Input: part model. Units: mm. Frame: model coordinates. A direction names the side the tool comes from. Coordinates: 2 decimals unless noted, no trailing zeros. Order: outer loops, then holes, each group sorted by start corner. A loop starts at its lowest first (then second) coordinate and runs counter-clockwise, first axis right, second up. Notation, with made-up numbers: (80.25, 5) -> (97.25, 5) arc R22 ccw to (97.25, 16) -> close; hole circle Ø2 at (78.25, 62.25). An arc over 180 degrees is marked (long way). Answer as CSV lines item,"result".
from build123d import *

# Parameters (mm, degrees)
SKETCH_1_R              = 19.5
EXTRUDE_1_DEPTH         = 25
CUT_EXTRUDE_1_DEPTH     = 5.95
SKETCH_3_R              = 20
EXTRUDE_2_DEPTH         = 21
SKETCH_4_R              = 23
EXTRUDE_3_DEPTH         = 150
CUT_EXTRUDE_START       = -30
CUT_EXTRUDE_2_DEPTH     = 30
HOLE_WIZARD_M10_1_D     = 8.5
HOLE_WIZARD_M10_1_DEPTH = 20
HOLE_WIZARD_M10_1_TIP   = 2.553657631


with BuildPart() as part:
    # 草图1 → 凸台-拉伸1 (new body)
    with BuildSketch(Plane(origin=(0, 0, 0), x_dir=(0, 0, -1), z_dir=(1, 0, 0))):
        Circle(SKETCH_1_R)
    extrude(amount=EXTRUDE_1_DEPTH)

    # 草图2 → 切除-拉伸1 (cut)
    with BuildSketch(Plane(origin=(0, 19.5, 0), x_dir=(1, 0, 0), z_dir=(0, 1, 0))):
        with BuildLine():
            Line((9, 6), (17, 6))
            ThreePointArc((17, 6), (23, 0), (17, -6))
            Line((17, -6), (9, -6))
            ThreePointArc((9, -6), (3, 0), (9, 6))
        make_face()
    extrude(amount=-CUT_EXTRUDE_1_DEPTH, mode=Mode.SUBTRACT)

    # 草图3 → 凸台-拉伸2 (add)
    with BuildSketch(Plane.ZY):
        with Locations(Location((0, 0, 0), (0, 0, 180))):
            Circle(SKETCH_3_R)
    extrude(amount=EXTRUDE_2_DEPTH)

    # 草图4 → 凸台-拉伸3 (add)
    with BuildSketch(Plane.ZY.offset(21)):
        Circle(SKETCH_4_R)
    extrude(amount=EXTRUDE_3_DEPTH)

    # 草图5 → 切除-拉伸2 (cut)
    with BuildSketch(Plane.ZY.offset(171).offset(CUT_EXTRUDE_START)):
        with BuildLine():
            ThreePointArc((18.852862485, -13.174580681), (21.255112475, -8.78750213), (22.652173913, -3.98484843))
            Line((22.652173913, -3.98484843), (20.658042319, -3.98484843))
            ThreePointArc((20.658042319, -3.98484843), (19.443275073, -8.036963599), (17.442433123, -11.764151318))
            Line((17.442433123, -11.764151318), (18.852862485, -13.174580681))
        make_face()
        with BuildLine():
            ThreePointArc((22.646822247, 4.01515157), (21.243336512, 8.81593182), (18.83521913, 13.199792435))
            Line((18.83521913, 13.199792435), (17.425155157, 11.789728463))
            ThreePointArc((17.425155157, 11.789728463), (19.431463114, 8.065480192), (20.652173913, 4.01515157))
            Line((20.652173913, 4.01515157), (22.646822247, 4.01515157))
        make_face()
        with BuildLine():
            Line((-20.652173913, -4.01515157), (-22.646822247, -4.01515157))
            ThreePointArc((-22.646822247, -4.01515157), (-21.243336512, -8.81593182), (-18.83521913, -13.199792435))
            Line((-18.83521913, -13.199792435), (-17.425155157, -11.789728463))
            ThreePointArc((-17.425155157, -11.789728463), (-19.431463114, -8.065480192), (-20.652173913, -4.01515157))
        make_face()
        with BuildLine():
            Line((-11.764151318, -17.442433123), (-13.174580681, -18.852862485))
            ThreePointArc((-13.174580681, -18.852862485), (-8.78750213, -21.255112475), (-3.98484843, -22.652173913))
            Line((-3.98484843, -22.652173913), (-3.98484843, -20.658042319))
            ThreePointArc((-3.98484843, -20.658042319), (-8.036963599, -19.443275073), (-11.764151318, -17.442433123))
        make_face()
        with BuildLine():
            ThreePointArc((4.01515157, -22.646822247), (8.81593182, -21.243336512), (13.199792435, -18.83521913))
            Line((13.199792435, -18.83521913), (11.789728463, -17.425155157))
            ThreePointArc((11.789728463, -17.425155157), (8.065480192, -19.431463114), (4.01515157, -20.652173913))
            Line((4.01515157, -20.652173913), (4.01515157, -22.646822247))
        make_face()
        with BuildLine():
            ThreePointArc((13.174580681, 18.852862485), (8.78750213, 21.255112475), (3.98484843, 22.652173913))
            Line((3.98484843, 22.652173913), (3.98484843, 20.658042319))
            ThreePointArc((3.98484843, 20.658042319), (8.036963599, 19.443275073), (11.764151318, 17.442433123))
            Line((11.764151318, 17.442433123), (13.174580681, 18.852862485))
        make_face()
        with BuildLine():
            Line((-4.01515157, 20.652173913), (-4.01515157, 22.646822247))
            ThreePointArc((-4.01515157, 22.646822247), (-8.81593182, 21.243336512), (-13.199792435, 18.83521913))
            Line((-13.199792435, 18.83521913), (-11.789728463, 17.425155157))
            ThreePointArc((-11.789728463, 17.425155157), (-8.065480192, 19.431463114), (-4.01515157, 20.652173913))
        make_face()
        with BuildLine():
            Line((-17.442433123, 11.764151318), (-18.852862485, 13.174580681))
            ThreePointArc((-18.852862485, 13.174580681), (-21.255112475, 8.78750213), (-22.652173913, 3.98484843))
            Line((-22.652173913, 3.98484843), (-20.658042319, 3.98484843))
            ThreePointArc((-20.658042319, 3.98484843), (-19.443275073, 8.036963599), (-17.442433123, 11.764151318))
        make_face()
    extrude(amount=CUT_EXTRUDE_2_DEPTH, mode=Mode.SUBTRACT)

    # M10 螺纹孔1
    with Locations(Plane(origin=(25, 0, 0), x_dir=(0, 0, -1), z_dir=(1, 0, 0))):
        with Locations((0, 0)):
            Hole(HOLE_WIZARD_M10_1_D / 2, depth=HOLE_WIZARD_M10_1_DEPTH)
            with Locations((0, 0, -(HOLE_WIZARD_M10_1_DEPTH + HOLE_WIZARD_M10_1_TIP / 2))):  # 118° drill point
                Cone(0, HOLE_WIZARD_M10_1_D / 2, HOLE_WIZARD_M10_1_TIP, mode=Mode.SUBTRACT)


solid = part.part
1. Cut plane C-C (x = -111). Return the cut outline in (y, z), plus the area to 3 significant figures.
Findings:
outline,"circle Ø46 at (0, 0)"
area,"1,660 mm2"
2. Cut plane D-D (x = -10.5). Return the cut outline in (y, z), plus the area to 3 significant figures.
Findings:
outline,"circle Ø40 at (0, 0)"
area,"1,260 mm2"
3. Reachability of faces 5 (the face through (0, 4.4, -19.2)), 6 (the face through (-171, 0, 0)), 7 (the face through (-155.79, 7.982, -19.466)), 8 (the face through (-155.79, 19.41, -8.12)), 9 (the face through (3, 17, 0)) from +Z, -Z, +X, -X, +Y, -Y: full face, straight path, thin tool, end or side. Return the list, or none.
Findings:
face 5,"+X"
face 6,"+Z, -Z, -X, +Y, -Y"
face 7,"-Z, -X"
face 8,"-X, +Y"
face 9,"+Y"
4. Cut plane B-B (y = -10). Return the cut outline in (x, z).
Findings:
outline,"(-171, -18.51) -> (-141, -18.51) -> (-141, -20.71) -> (-21, -20.71) -> (-21, -17.32) -> (0, -17.32) -> (0, -16.74) -> (25, -16.74) -> (25, 16.74) -> (0, 16.74) -> (0, 17.32) -> (-21, 17.32) -> (-21, 20.71) -> (-141, 20.71) -> (-141, 18.51) -> (-171, 18.51) -> close"
5. Contact query for flat-ended pins moving along their axis: pin 1 (5 mm diameter, centred on y = 0, z = 0, fed in from +X); pin 2 (0.6 mm diameter, centred on x = -149, z = 21, fed in from -Y); pin 3 (1.6 mm diameter, centred on x = -161, z = 22, fed in from +Y). Output: stop coordinate, or through.
Findings:
pin 1,"stops at x = 3.95"
pin 2,"stops at y = -3.98"
pin 3,"stops at y = 4.02"
6. Mould query, pull axis Z, two halves, no side actions, for faces 1 (the face through (23, 17, 0)), 2 (the face through (25, 5, 0)), 3 (the face through (-155.79, -7.982, 19.466)), 4 (the face through (-94.95, 15.544, -16.952)). Classes: released by +Z, released by -Z, zero draft, split by the parting line, or undercut.
Findings:
face 1,"undercut"
face 2,"zero draft"
face 3,"released by +Z"
face 4,"split by the parting line"
7. Ray query, line 1 along Y through (x, z) = (15, 0); line 2 along Z through (x, y) = (-37, 4); line 3 along Z through (x, y) = (-136, -1). Return the intervals inside material, ascending.
Findings:
line 1,"y = -19.5 to -4.25, 4.25 to 13.55"
line 2,"z = -22.65 to 22.65"
line 3,"z = -22.98 to 22.98"
